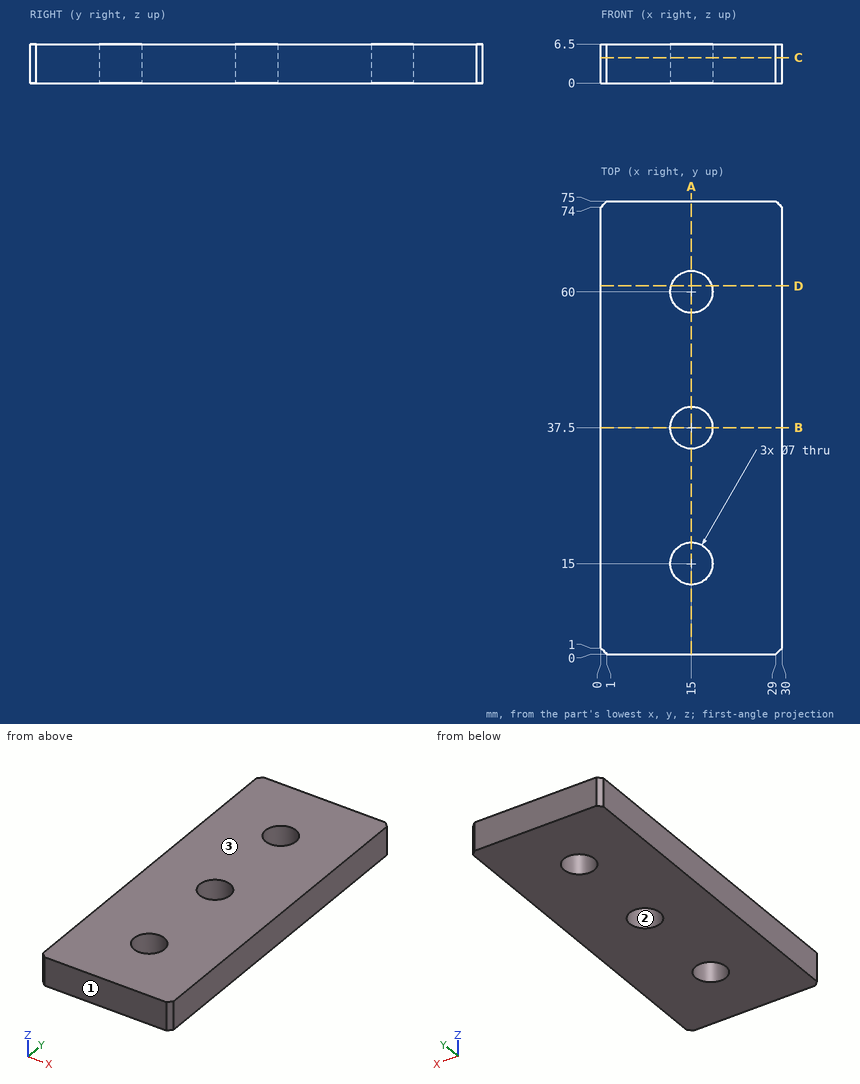
Can you work these out from the drawing? Everything is in mm from the part's minimum corner. Coordinates: 2 decimals unless noted, no trailing zeros. Loops run counter-clockwise (first coordinate to the right, second up) from the corner with the lowest first, then second, coordinate; pieces in that order, holes last. Notation, with made-up numbers: (19.5, -14) -> (50.5, -14) arc R18 ccw to (50.5, 5) -> close; hole circle Ø2 at (15.5, -3). An arc over 180 degrees is marked (long way). Return JSON: item names as keys, results as strings.
1) Thinking about a two-plate mould opening in Y: for the marked faces 1, 2 and 3, which applies, +Y half, -Y half, draft (parallel to the pull), parting line (faces both ways), or undercut?
Results below:
{"face 1": "-Y half", "face 2": "undercut", "face 3": "draft"}
2) If we section it at B-B, the plane y = 37.5: Write out the boundary of the cut face in (x, z).
Results below:
{"outline": "(0, 0) -> (11.5, 0) -> (11.5, 6.5) -> (0, 6.5) -> close; (18.5, 0) -> (30, 0) -> (30, 6.5) -> (18.5, 6.5) -> close"}
3) If we section it at A-A, the plane x = 15: Write out the boundary of the cut face in (y, z).
Results below:
{"outline": "(0, 0) -> (11.5, 0) -> (11.5, 6.5) -> (0, 6.5) -> close; (18.5, 0) -> (34, 0) -> (34, 6.5) -> (18.5, 6.5) -> close; (41, 0) -> (56.5, 0) -> (56.5, 6.5) -> (41, 6.5) -> close; (63.5, 0) -> (75, 0) -> (75, 6.5) -> (63.5, 6.5) -> close"}
4) If we section it at C-C, the plane z = 4.25: Write out the boundary of the cut face in (x, y), then the cut area to 3 significant figures.
Results below:
{"outline": "(0, 1) -> (1, 0) -> (29, 0) -> (30, 1) -> (30, 74) -> (29, 75) -> (1, 75) -> (0, 74) -> close; hole circle Ø7 at (15, 15); hole circle Ø7 at (15, 37.5); hole circle Ø7 at (15, 60)", "area": "2,130 mm²"}
5) I need wall thicknesses on line 1 (Y direction, x = 15, z = 4.5); line 2 (X direction, y = 61.5, z = 5); line 3 (X direction, y = 12.5, z = 5.5). Which ranges of each line are inside material? Lowest first, please. Write a range as from..to.
Results below:
{"line 1": "0..11.5, 18.5..34, 41..56.5, 63.5..75", "line 2": "0..11.84, 18.16..30", "line 3": "0..12.55, 17.45..30"}
6) If we section it at D-D, the plane y = 61: Write out the boundary of the cut face in (x, z), then the cut area to 3 significant figures.
Results below:
{"outline": "(0, 0) -> (11.65, 0) -> (11.65, 6.5) -> (0, 6.5) -> close; (18.35, 0) -> (30, 0) -> (30, 6.5) -> (18.35, 6.5) -> close", "area": "151 mm²"}
7) Will this pin go through, and if not, where does the flat tip stop? pin 1 (9 mm diameter, centred on x = 15, y = 37.5, fed in from -Z).
Results below:
{"pin 1": "z = 0"}
